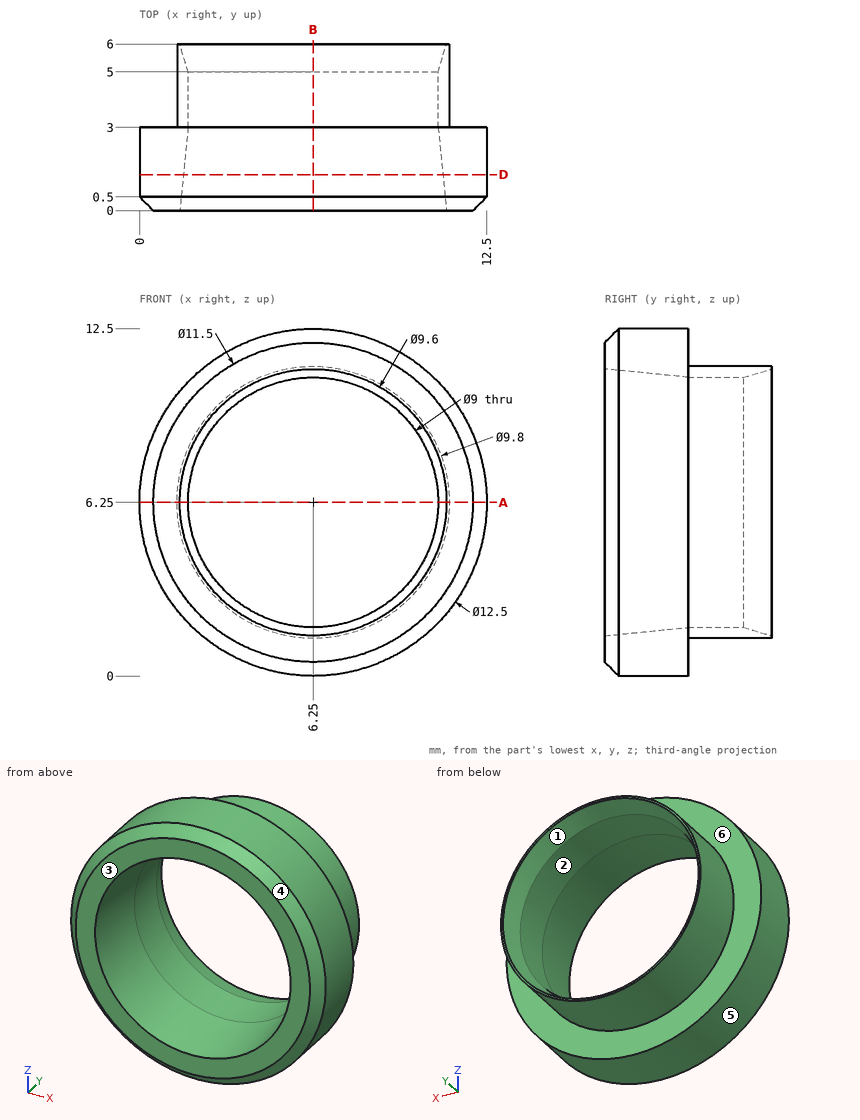
The figure shows three views and two pictorial views of one solid part (mm, origin at its lowest corner). Answer the questions. A direction names the side the tool comes from. Round coordinates to 2 decimals unless told otherwise and drop trailing zeros. Write each loop counter-clockwise with the first axis right and the second up, starting at its lowest first coordinate (ties: lowest second). Pieces come first, ordered by that corner, then holes. Notation, with made-up numbers: (66, 74) - (97, 74) arc R22 cw to (97, 94) - close; hole circle Ø6 at (0, -16). An arc over 180 degrees is marked (long way). Use one line per item in the form item = value. Start each with the question number.
Item 1: Flat-ended cylindrical pins translate along their axes: pin 1 Ø2 at (y, z) = (2.5, 9) entering from -X; pin 2 Ø1.5 at (y, z) = (2, 10) entering from -X; pin 3 Ø2 at (y, z) = (3.5, 10) entering from +X. Find the tip coordinate at first contact, or state that the pin passes through.
Item 2: A cutting plane is placed at D-D (y = 1.3). Write down the section's boundary in (x, z), plus the area to 3 significant figures.
Item 3: A cutting plane is placed at B-B (x = 6.25). Write down the section's boundary in (y, z).
Item 4: A cutting plane is placed at A-A (z = 6.25). Write down the section's boundary in (x, y), plus the area to 4 significant figures.
Item 5: Find the intervals of material crossed by line 1 (X direction, y = 3.45, z = 6.25); line 2 (Y direction, x = 9.5, z = 10); line 3 (Z direction, x = 8, y = 4.3), in increasing order. Write a range as [from, to].
Item 6: A tool of negligible diameter and unlimited length cuts with its end or side. For the marked faces 5 and 6, from which of +Z, -Z, +X, -X, +Y, -Y can it reach the whole face along a straight path? Write none if from no direction.
Item 7: Determine the mould class of the marked faces 1, 2, 3 and 4 for opening direction Z: +Z half, -Z half, draft (parallel to the pull), parting line (faces both ways), or undercut.
The answers:
q1.pin_1 = 0.25
q1.pin_2 = 0.77
q1.pin_3 = 11.79
q2.outline = circle Ø12.5 at (6.25, 6.25); hole circle Ø9.34 at (6.25, 6.25)
q2.area = 54.2 mm^2
q3.outline = (0, 0.5) - (0.5, 0) - (3, 0) - (3, 1.35) - (6, 1.35) - (6, 1.45) - (5, 1.75) - (3, 1.75) - (0, 1.45) - close; (0, 11.05) - (3, 10.75) - (5, 10.75) - (6, 11.05) - (6, 11.15) - (3, 11.15) - (3, 12.5) - (0.5, 12.5) - (0, 12) - close
q4.outline = (0, 0.5) - (0.5, 0) - (1.45, 0) - (1.75, 3) - (1.75, 5) - (1.45, 6) - (1.35, 6) - (1.35, 3) - (0, 3) - close; (10.75, 3) - (11.05, 0) - (12, 0) - (12.5, 0.5) - (12.5, 3) - (11.15, 3) - (11.15, 6) - (11.05, 6) - (10.75, 5) - close
q4.area = 11.45 mm^2
q5.line_1 = [1.35, 1.75], [10.75, 11.15]
q5.line_2 = [0, 3]
q5.line_3 = [1.67, 2.1], [10.4, 10.83]
q6.face_5 = +Y, -Y
q6.face_6 = +Y
q7.face_1 = undercut
q7.face_2 = undercut
q7.face_3 = draft
q7.face_4 = parting line
